```python
from build123d import *

# Parameters (mm, degrees)
SKETCH_1_W                = 160
SKETCH_1_H                = 80
EXTRUDE_1_DEPTH           = 12
HOLE_WIZARD_M8_1_D        = 6.8
HOLE_WIZARD_1_D           = 5.5
HOLE_WIZARD_1_CBORE_D     = 10
HOLE_WIZARD_1_CBORE_DEPTH = 5.7


with BuildPart() as part:
    # 草图1 → 凸台-拉伸1 (new body)
    with BuildSketch(Plane(origin=(0, 0, 0), x_dir=(0, 0, -1), z_dir=(1, 0, 0))):
        Rectangle(SKETCH_1_W, SKETCH_1_H)
    extrude(amount=EXTRUDE_1_DEPTH)

    # M8 螺纹孔1 (through all)
    with Locations(Plane(origin=(12, 0, 0), x_dir=(0, 0, -1), z_dir=(1, 0, 0))):
        with Locations((-70, 14), (-70, -14), (-26, 14), (-26, -14)):
            Hole(HOLE_WIZARD_M8_1_D / 2)

    # 打孔尺寸(%根据)内六角圆柱头螺钉的类型1 (through all)
    with Locations(Plane(origin=(12, 0, 0), x_dir=(0, 0, -1), z_dir=(1, 0, 0))):
        with Locations((-60, 14), (-60, -14), (60, 14), (60, -14)):
            CounterBoreHole(HOLE_WIZARD_1_D / 2, HOLE_WIZARD_1_CBORE_D / 2, HOLE_WIZARD_1_CBORE_DEPTH)


solid = part.part
```
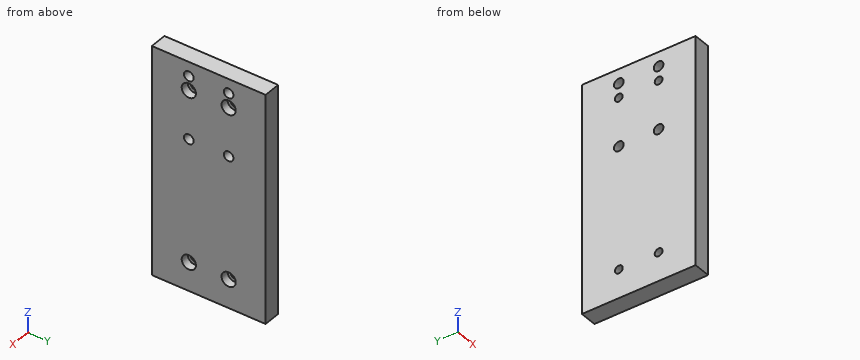
Part model, mm, in its own coordinate system. Round coordinates to 2 decimals unless told otherwise and drop trailing zeros. Write each loop counter-clockwise with the first axis right and the second up, starting at its lowest first coordinate (ties: lowest second). Pieces come first, ordered by that corner, then holes.
Item 1: Drop flat-ended pins along their axis: pin 1 Ø5.5 at (y, z) = (-14, 70) entering from +X; pin 2 Ø3 at (y, z) = (12, -58) entering from +X; pin 3 Ø11 at (y, z) = (14, 61) entering from +X. Give the stop position or say it passes through.
Results:
pin 1: passes through
pin 2: stops at x = 6.3
pin 3: stops at x = 12
Item 2: Probe L1, parallel to Y at x = 10, z = 60; L2, parallel to Y at x = 8.25, z = 26; L3, parallel to Z at x = 1.5, y = -15.5. List the from-to ranges inside material, lowest first.
Results:
L1: y = -40 to -19, -9 to 9, 19 to 40
L2: y = -40 to -17.4, -10.6 to 10.6, 17.4 to 40
L3: z = -80 to -62.3, -57.7 to 22.95, 29.05 to 57.7, 62.3 to 66.95, 73.05 to 80
Item 3: Cut at C-C, the plane x = 9. Count the separate pieces of the cut face and the enclosed holes in it, plus the area to 3 significant figures.
Results:
separate pieces: 1
enclosed holes: 8
area: 12,300 mm2
Item 4: Cut at B-B, the plane y = -14. Give the cut face in (x, z), plus the area to 3 significant figures.
Results:
outline: (0, -80) - (12, -80) - (12, -65) - (6.3, -65) - (6.3, -62.75) - (0, -62.75) - close; (0, -57.25) - (6.3, -57.25) - (6.3, -55) - (12, -55) - (12, 22.6) - (0, 22.6) - close; (0, 29.4) - (12, 29.4) - (12, 55) - (6.3, 55) - (6.3, 57.25) - (0, 57.25) - close; (0, 62.75) - (6.3, 62.75) - (6.3, 65) - (12, 65) - (12, 66.6) - (0, 66.6) - close; (0, 73.4) - (12, 73.4) - (12, 80) - (0, 80) - close
area: 1,570 mm2
Item 5: Cut at A-A, the plane z = 70. Give the cut face in (x, y).
Results:
outline: (0, -40) - (12, -40) - (12, -17.4) - (0, -17.4) - close; (0, -10.6) - (12, -10.6) - (12, 10.6) - (0, 10.6) - close; (0, 17.4) - (12, 17.4) - (12, 40) - (0, 40) - close
Item 6: Cut at D-D, the plane z = -60. Give the cut face in (x, y), plus the area to 3 significant figures.
Results:
outline: (0, -40) - (12, -40) - (12, -19) - (6.3, -19) - (6.3, -16.75) - (0, -16.75) - close; (0, -11.25) - (6.3, -11.25) - (6.3, -9) - (12, -9) - (12, 9) - (6.3, 9) - (6.3, 11.25) - (0, 11.25) - close; (0, 16.75) - (6.3, 16.75) - (6.3, 19) - (12, 19) - (12, 40) - (0, 40) - close
area: 777 mm2
